Geometry: final body of the model. Coordinates: model frame, mm. Face numbers are marked on the shaded views. A direction names the side the tool comes from. Give positions to 0.01 mm unless a question says otherwise; leave off trailing zeros. Order: outer loops, then holes, each group sorted by start corner. A loop starts at its lowest first (then second) coordinate and runs counter-clockwise, first axis right, second up. Notation, with made-up numbers: (-2.75, 15) - (51.25, 15) arc R23 cw to (51.25, 54) - close; hole circle Ø8 at (45.5, 89.5). An arc over 180 degrees is marked (long way). One line per question, with ' | ' between items. Start each with the question number.
from build123d import *

# Parameters (mm, degrees)
SQUARE_BAR_20X82_DEPTH          = 82
TOP_POCKET_PROFILE_19_R         = 9.5
TOP_POCKET_19X5_DEPTH           = 5
END_SPIGOT_PROFILE_20_R         = 10
END_SPIGOT_20X15_DEPTH          = 15
SKETCH3_3_R                     = 6
SPIGOT_CONTOUR_TRIM_CUT_DEPTH   = 85.403791384
CROSS_TAPPED_HOLE_1_4_28_REACH  = 95.771
CROSS_TAPPED_HOLE_1_4_28_BORE_R = 2.7051


with BuildPart() as part:
    # Square Bar Profile 20 → Square Bar 20x82 (new body)
    with BuildSketch(Plane(origin=(0, 0, 0), x_dir=(1, 0, 0), z_dir=(0, 1, 0))):
        Polygon((-14.142135624, 0), (0, 14.142135624), (14.142135624, 0), (0, -14.142135624), align=None)
    extrude(amount=SQUARE_BAR_20X82_DEPTH)

    # Top Pocket Profile _19 → Top Pocket _19x5 (cut)
    with BuildSketch(Plane(origin=(0, 82, 0), x_dir=(1, 0, 0), z_dir=(0, 1, 0))):
        with Locations(Location((0, 0, 0), (0, 0, 270))):
            Circle(TOP_POCKET_PROFILE_19_R)
    extrude(amount=-TOP_POCKET_19X5_DEPTH, mode=Mode.SUBTRACT)

    # End Spigot Profile _20 → End Spigot _20x15 (add)
    with BuildSketch(Plane.XZ):
        with Locations(Location((0, 0, 0), (0, 0, 45))):
            Circle(END_SPIGOT_PROFILE_20_R)
    extrude(amount=END_SPIGOT_20X15_DEPTH)

    # Sketch3_3 → Spigot Contour Trim Cut (cut, through all)
    with BuildSketch(Plane.XZ):
        with Locations(Location((0, 0, 0), (0, 0, 270))):
            Circle(SKETCH3_3_R)
    extrude(amount=SPIGOT_CONTOUR_TRIM_CUT_DEPTH, mode=Mode.SUBTRACT)

    # Cross Tapped Hole 1-4-28 bore (on position points) → Cross Tapped Hole 1-4-28 (cut, up to next)
    with BuildSketch(Plane(origin=(0, -7.5, 10), x_dir=(1, 0, 0), z_dir=(0, 0, 1)), mode=Mode.PRIVATE) as cross_tapped_hole_1_4_28_sk1:
        Circle(CROSS_TAPPED_HOLE_1_4_28_BORE_R)
    cross_tapped_hole_1_4_28_tool1 = extrude(cross_tapped_hole_1_4_28_sk1.sketch, amount=-CROSS_TAPPED_HOLE_1_4_28_REACH, mode=Mode.PRIVATE) & part.part
    add(cross_tapped_hole_1_4_28_tool1.solids().sort_by_distance((0, -7.5, 10))[0], mode=Mode.SUBTRACT)


solid = part.part
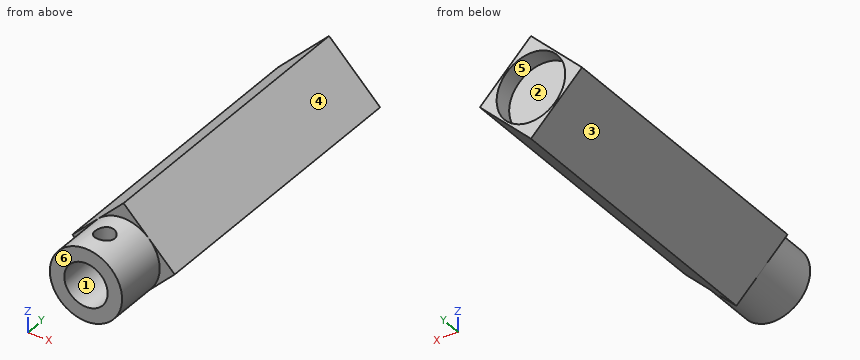
(1) Cut plane C-C, the plane y = 19. Return the cut outline in (x, z), plus the area to 3 significant figures.
(2) Cut plane A-A, the plane x = 1.25. Return the cut outline in (y, z), plus the area to 3 significant figures.
(3) Material intervals for line 1 along Y through (x, z) = (0, 8.5); line 2 along Z through (x, y) = (0, -3.5), sorted ascending. Write a range as from..to.
(4) Pull-direction query (X, two-part tool) for the marked faces 4, 5 and 6; classes: +X half, -X half, draft (parallel to the pull), parting line (faces both ways), or undercut.
(5) Cut plane D-D, the plane z = -11.25. Return the cut outline in (x, y), plus the area to 3 significant figures.
(6) Contact query for flat-ended pins moving along their axis: P1, Ø2, axis at y = 62, z = -6.5, coming from the -X side; P2, Ø1.5, axis at x = -7, y = 69, coming from the +Z side; P3, Ø5, axis at x = 5.5, y = 17, coming from the +Z side; P4, Ø14, axis at x = 0, z = 0, coming from the -Y side. Output: stop coordinate, or through.
(7) Cut plane B-B, the plane z = -1.5. Return the cut outline in (x, y).
(8) Access query for the marked faces 1, 2 and 3. Directions: +Z, -Z, +X, -X, +Y, -Y. A direction counts if a zero-diameter tool reaches every point of the face in a straight line with its end or side. Return the directions, or none.
Results are:
1) outline: (-14.14, 0) - (0, -14.14) - (14.14, 0) - (0, 14.14) - close | area: 400 mm2
2) outline: (-15, -9.92) - (0, -9.92) - (0, -12.89) - (82, -12.89) - (82, -9.42) - (77, -9.42) - (77, 9.42) - (82, 9.42) - (82, 12.89) - (0, 12.89) - (0, 9.92) - (-5.1, 9.92) - (-5.1, 5.87) - (0, 5.87) - (0, -5.87) - (-15, -5.87) - close; (-15, 5.87) - (-9.9, 5.87) - (-9.9, 9.92) - (-15, 9.92) - close | area: 2,120 mm2
3) line 1: -15..-10.21, -4.79..77 | line 2: -10..-6, 6..10
4) face 4: +X half | face 5: undercut | face 6: draft
5) outline: (-2.89, 0) - (2.89, 0) - (2.89, 82) - (-2.89, 82) - close | area: 474 mm2
6) P1: x = -8.64 | P2: z = 7.89 | P3: z = 11.14 | P4: y = -15
7) outline: (-12.64, 0) - (-9.89, 0) - (-9.89, -15) - (-5.81, -15) - (-5.81, 0) - (5.81, 0) - (5.81, -15) - (9.89, -15) - (9.89, 0) - (12.64, 0) - (12.64, 82) - (9.38, 82) - (9.38, 77) - (-9.38, 77) - (-9.38, 82) - (-12.64, 82) - close
8) face 1: -Y | face 2: +Y | face 3: -Z, -X, +Y, -Y
